from build123d import *

# Parameters (mm, degrees)
BRACKET_BODY_DEPTH         = 90
ANGLED_CUT_DEPTH           = 25
ARM_BOSS_SKETCH_R          = 7.5
ARM_BOSS_DEPTH             = 15
CORNER_FILLETS_R10_R       = 10
CORNER_HOLES_10_DEPTH      = 202.651164925
CORNER_HOLES_10_DEPTH_BACK = 202.651164925
CORNER_HOLES_SKETCH_R      = 5
FACE_HOLES_2X_8_DEPTH      = 168.107749671
FACE_HOLES_2X_8_DEPTH_BACK = 168.107749671
FACE_HOLES_SKETCH_R        = 4


with BuildPart() as part:
    # Bracket Profile Sketch → Bracket Body (new body)
    with BuildSketch(Plane(origin=(0, 0, 0), x_dir=(1, 0, 0), z_dir=(0, 1, 0))):
        Polygon((-24, -7.5), (-24, -32.5), (-40, -32.5), (-40, 7.5), (-24, 7.5), (40, 7.5), (40, -7.5), align=None)
    extrude(amount=BRACKET_BODY_DEPTH)

    # Angled Cut Sketch → Angled Cut (cut)
    with BuildSketch(Plane(origin=(0, 90, 0), x_dir=(1, 0, 0), z_dir=(0, 1, 0))):
        Polygon((40, 7.5), (25, 7.5), (40, -7.5), align=None)
    angled_cut = extrude(amount=-ANGLED_CUT_DEPTH, mode=Mode.SUBTRACT)

    # Angled Cut Mirror: Angled Cut across plane
    add(angled_cut.mirror(Plane.ZX.offset(45)), mode=Mode.SUBTRACT)

    # Arm Boss Sketch → Arm Boss (add, symmetric)
    with BuildSketch(Plane(origin=(0, 45, 0), x_dir=(1, 0, 0), z_dir=(0, 1, 0))):
        with BuildLine():
            Line((40, -7.5), (135, -7.5))
            Line((135, -7.5), (135, 29.024905628))
            ThreePointArc((135, 29.024905628), (120, 44.024905628), (105, 29.024905628))
            Line((105, 29.024905628), (105, 7.5))
            Line((105, 7.5), (40, 7.5))
            Line((40, 7.5), (40, -7.5))
        make_face()
        with Locations(Location((120, 29.024905628, 0), (0, 0, 270))):
            Circle(ARM_BOSS_SKETCH_R, mode=Mode.SUBTRACT)
    extrude(amount=ARM_BOSS_DEPTH, both=True)

    # Corner Fillets R10
    corner_fillets_r10_edges = [part.edges().sort_by_distance(p)[0] for p in [
        (-32, 90, 32.5),
        (-32, 0, 32.5),
    ]]
    fillet(corner_fillets_r10_edges, radius=CORNER_FILLETS_R10_R)

    # Corner Holes Sketch → Corner Holes Ø10 (cut, two sides: drawn at the far end of the back side and taken through both)
    with BuildSketch(Plane.ZY.offset(40).offset(-CORNER_HOLES_10_DEPTH_BACK)):
        with Locations((22.5, 80)):
            Circle(CORNER_HOLES_SKETCH_R)
        with Locations((22.5, 10)):
            Circle(CORNER_HOLES_SKETCH_R)
    extrude(amount=CORNER_HOLES_10_DEPTH + CORNER_HOLES_10_DEPTH_BACK, mode=Mode.SUBTRACT)

    # Face Holes Sketch → Face Holes 2xØ8 (cut, two sides: drawn at the far end of the back side and taken through both)
    with BuildSketch(Plane(origin=(0, 0, -7.5), x_dir=(-1, 0, 0), z_dir=(0, 0, -1)).offset(-FACE_HOLES_2X_8_DEPTH_BACK)):
        with Locations((10, 45)):
            Circle(FACE_HOLES_SKETCH_R)
        with Locations((-15, 45)):
            Circle(FACE_HOLES_SKETCH_R)
    extrude(amount=FACE_HOLES_2X_8_DEPTH + FACE_HOLES_2X_8_DEPTH_BACK, mode=Mode.SUBTRACT)


solid = part.part
Verification items for the finished model (mm, model axes). A direction names the side the tool comes from. Coordinates: 2 decimals unless noted, no trailing zeros. Loops run counter-clockwise (first coordinate to the right, second up) from the corner with the lowest first, then second, coordinate; pieces in that order, holes last. Notation, with made-up numbers: (8, 80) -> (14, 80) arc R20 ccw to (14, 102) -> close; hole circle Ø11 at (13, 39). An arc over 180 degrees is marked (long way). Answer as a JSON object with one key per item and string values. Group by question number.
Item 1: Depth check by flat-ended pin: pin 1 (10.5 mm diameter, centred on x = -10, y = 45, fed in from +Z); pin 2 (12.5 mm diameter, centred on y = 60.5, z = 20.5, fed in from +X); pin 3 (7 mm diameter, centred on x = 15, y = 45, fed in from +Z); pin 4 (4 mm diameter, centred on y = 62.5, z = -2, fed in from +X). Enter the tip coordinate at first touch or a pass-through.
Item 2: Sectioned sample at C-C on y = 35. Record the boundary of the cut face in (x, z), plus the area to 3 significant figures.
Item 3: Scan lines: probe 1 along Y at (x, z) = (-36, 22.5); probe 2 along X at (y, z) = (45, 1.75); probe 3 along Z at (x, y) = (-29, 80). Record each from-to range of solid material in increasing order.
Item 4: Tool access check on faces 5 (the flat face through (36, 65, -3)), 6 (the flat face through (17, 54, -7.5)), 7 (the flat face through (40, 27, 0)), 8 (the flat face through (32.4, 12.3, -0.1)), 9 (the flat face through (-24, 44, 20)). Record the directions out of +Z, -Z, +X, -X, +Y, -Y that give a thin tool (end or side, any length) a straight path to the whole face; none if there is none.
Item 5: Sectioned sample at D-D on z = 20. Record the boundary of the cut face in (x, y), plus the area to 3 significant figures.
Item 6: Sectioned sample at A-A on x = 120. Record the boundary of the cut face in (y, z).
Item 7: Sectioned sample at B-B on x = -27. Record the boundary of the cut face in (y, z).
Item 8: Mould release check, pull along Y, two halves, no side actions. Record for faces 1 (the flat face through (97, 60, -7)), 2 (the flat face through (97, 30, -7)), 3 (the cylindrical face through (-31.888, 13.379, 18.815)), 4 (the flat face through (40, 62, 0)): +Y half, -Y half, draft (parallel to the pull), parting line (faces both ways), or undercut.
Evaluation:
{
 "1": {"pin 1": "stops at z = 7.5", "pin 2": "stops at x = -24", "pin 3": "passes through", "pin 4": "stops at x = 40"},
 "2": {"outline": "(-40, -7.5) -> (105, -7.5) -> (105, -29.02) arc R15 ccw to (135, -29.02) -> (135, 7.5) -> (-24, 7.5) -> (-24, 32.5) -> (-40, 32.5) -> close; hole circle Ø15 at (120, -29.02)", "area": "3,850 mm²"},
 "3": {"probe 1": "y = 0 to 5, 15 to 75, 85 to 90", "probe 2": "x = -40 to -14, -6 to 11, 19 to 135", "probe 3": "z = -7.5 to 17.5, 27.5 to 32.5"},
 "4": {"face 5": "-Z, +X, +Y", "face 6": "-Z, -X, +Y, -Y", "face 7": "+Z, -Z, +X, -Y", "face 8": "-Z, +X, -Y", "face 9": "+Z, +X, +Y, -Y"},
 "5": {"outline": "(-40, 0) -> (-24, 0) -> (-24, 5.67) -> (-40, 5.67) -> close; (-40, 14.33) -> (-24, 14.33) -> (-24, 75.67) -> (-40, 75.67) -> close; (-40, 84.33) -> (-24, 84.33) -> (-24, 90) -> (-40, 90) -> close", "area": "1,160 mm²"},
 "6": {"outline": "(30, -44.02) -> (60, -44.02) -> (60, -36.52) -> (30, -36.52) -> close; (30, -21.52) -> (60, -21.52) -> (60, 7.5) -> (30, 7.5) -> close"},
 "7": {"outline": "(0, -7.5) -> (90, -7.5) -> (90, 22.5) arc R10 ccw to (80, 32.5) -> (10, 32.5) arc R10 ccw to (0, 22.5) -> close; hole circle Ø10 at (10, 22.5); hole circle Ø10 at (80, 22.5)"},
 "8": {"face 1": "+Y half", "face 2": "-Y half", "face 3": "undercut", "face 4": "draft"}
}
